Here's how the part is built. I have some questions about the finished solid (model axes, mm). A direction names the side the tool comes from. Coordinates: 2 decimals unless noted, no trailing zeros. Order: outer loops, then holes, each group sorted by start corner. A loop starts at its lowest first (then second) coordinate and runs counter-clockwise, first axis right, second up.
```python
from build123d import *

# Parameters (mm, degrees)
BOSS_EXTRUDE1_DEPTH = 435
SKETCH2_R           = 8.5
CUT_EXTRUDE1_DEPTH  = 435
CUT_EXTRUDE2_DEPTH  = 435


with BuildPart() as part:
    # Sketch1 → Boss-Extrude1 (new body)
    with BuildSketch(Plane.XY):
        with BuildLine():
            Line((0, 0), (0, 40))
            ThreePointArc((0, 40), (2.928932188, 47.071067812), (10, 50))
            Line((10, 50), (90, 50))
            ThreePointArc((90, 50), (97.071067812, 47.071067812), (100, 40))
            Line((100, 40), (100, 0))
            Line((100, 0), (94, 0))
            Line((94, 0), (94, 40))
            ThreePointArc((94, 40), (92.828427125, 42.828427125), (90, 44))
            Line((90, 44), (10, 44))
            ThreePointArc((10, 44), (7.171572875, 42.828427125), (6, 40))
            Line((6, 40), (6, 0))
            Line((6, 0), (0, 0))
        make_face()
    extrude(amount=BOSS_EXTRUDE1_DEPTH)

    # Sketch2 → Cut-Extrude1 (cut)
    with BuildSketch(Plane(origin=(0, 50, 0), x_dir=(1, 0, 0), z_dir=(0, 1, 0))):
        with Locations(Location((73.2, -35.5, 0), (0, 0, 270))):
            Circle(SKETCH2_R)
    extrude(amount=-CUT_EXTRUDE1_DEPTH, mode=Mode.SUBTRACT)

    # Sketch3 → Cut-Extrude2 (cut)
    with BuildSketch(Plane(origin=(100, 0, 0), x_dir=(0, 0, -1), z_dir=(1, 0, 0))):
        Polygon((-80, 0), (0, 35), (0, 0), align=None)
    extrude(amount=-CUT_EXTRUDE2_DEPTH, mode=Mode.SUBTRACT)


solid = part.part
```
Q1. Will this pin go through, and if not, where does the flat tip stop? pin 1 (10 mm diameter, centred on x = 51, z = 170, fed in from -Y).
Q2. We'd pull the mould along Z, two halves only. Please class faces 3 (the cylindrical face through (64.9, 47.04, 33.66)), 4 (the flat face through (50, 45, 435)), 5 (the flat face through (94, 20, 214)): pulls with the +Z half, pulls with the -Z half, needs draft (parallel to the pull), parting line crosses it, or undercut.
Q3. If we section it at C-C on z = 35.5: Write out the boundary of the cut face in (x, y).
Q4. If we section it at D-D on z = 131: Write out the boundary of the cut face in (x, y).
Q5. I need wall thicknesses on L1, parallel to X at y = 36, z = 125; L2, parallel to Y at x = 53.5, z = 309; L3, parallel to X at y = 43, z = 289.5. Which ranges of each line are inside material? Lowest first, please.
Q6. If we section it at B-B on y = 21: Write out the boundary of the cut face in (x, z), then the cut area to 3 significant figures.
Q7. If we section it at A-A on x = 73.2: Write out the boundary of the cut face in (y, z), then the cut area to 3 significant figures.
Q8. For faces 1 (the flat face through (97.042, 17.255, 40.56)), 2 (the flat face through (51, 44, 214)), which set-ups out of +Z, -Z, +X, -X, +Y, -Y let a thin tool reach every point of the face, with its end or its side?
Reply:
1. pin 1: stops at y = 44
2. face 3: undercut
2. face 4: pulls with the +Z half
2. face 5: needs draft
3. outline: (0, 19.47) - (6, 19.47) - (6, 40) arc R4 cw to (10, 44) - (64.7, 44) - (64.7, 50) - (10, 50) arc R10 ccw to (0, 40) - close; (81.7, 44) - (90, 44) arc R4 cw to (94, 40) - (94, 19.47) - (100, 19.47) - (100, 40) arc R10 ccw to (90, 50) - (81.7, 50) - close
4. outline: (0, 0) - (6, 0) - (6, 40) arc R4 cw to (10, 44) - (90, 44) arc R4 cw to (94, 40) - (94, 0) - (100, 0) - (100, 40) arc R10 ccw to (90, 50) - (10, 50) arc R10 ccw to (0, 40) - close
5. L1: x = 0 to 6, 94 to 100
5. L2: y = 44 to 50
5. L3: x = 0.46 to 7.35, 92.65 to 99.54
6. outline: (0, 32) - (6, 32) - (6, 435) - (0, 435) - close; (94, 32) - (100, 32) - (100, 435) - (94, 435) - close
6. area: 4,840 mm2
7. outline: (44, 0) - (50, 0) - (50, 27) - (44, 27) - close; (44, 44) - (50, 44) - (50, 435) - (44, 435) - close
7. area: 2,510 mm2
8. face 1: -Z, +X, -X, -Y
8. face 2: +Z, -Z, -Y
